from build123d import *

# Parameters (mm, degrees)
BRACKET_PROFILE_DEPTH     = 6
UPRIGHT_ROUNDS_R5_R       = 5
BASE_PLATE_SKETCH_W       = 27
BASE_PLATE_SKETCH_H       = 6
BASE_PLATE_DEPTH          = 12
BASE_PLATE_ROUNDS_R6_R    = 6
BASE_UPRIGHT_FILLETS_R5_R = 5
BASE_SLOT_DEPTH           = 6
PIVOT_HOLES_SKETCH_R      = 2.5
PIVOT_HOLES_2X_5_DEPTH    = 6


with BuildPart() as part:
    # Bracket Profile Sketch → Bracket Profile (new body)
    with BuildSketch(Plane.XY):
        with BuildLine():
            Line((-20, 0), (20, 0))
            Line((20, 0), (20, 18))
            ThreePointArc((20, 18), (15, 23), (10, 18))
            Line((10, 18), (10, 6))
            Line((10, 6), (-10, 6))
            Line((-10, 6), (-10, 18))
            ThreePointArc((-10, 18), (-15, 23), (-20, 18))
            Line((-20, 18), (-20, 0))
        make_face()
    extrude(amount=BRACKET_PROFILE_DEPTH)

    # Upright Rounds R5
    upright_rounds_r5_edges = [part.edges().sort_by_distance(p)[0] for p in [
        (-10, 6, 3),
        (10, 6, 3),
    ]]
    fillet(upright_rounds_r5_edges, radius=UPRIGHT_ROUNDS_R5_R)

    # Base Plate Sketch → Base Plate (add)
    with BuildSketch(Plane.XY.offset(6)):
        with Locations((0, 3)):
            Rectangle(BASE_PLATE_SKETCH_W, BASE_PLATE_SKETCH_H)
    extrude(amount=BASE_PLATE_DEPTH)

    # Base Plate Rounds R6
    base_plate_rounds_r6_edges = [part.edges().sort_by_distance(p)[0] for p in [
        (-13.5, 3, 18),
        (13.5, 3, 18),
    ]]
    fillet(base_plate_rounds_r6_edges, radius=BASE_PLATE_ROUNDS_R6_R)

    # Base-Upright Fillets R5
    base_upright_fillets_r5_edges = [part.edges().sort_by_distance(p)[0] for p in [
        (-13.5, 3, 6),
        (13.5, 3, 6),
    ]]
    fillet(base_upright_fillets_r5_edges, radius=BASE_UPRIGHT_FILLETS_R5_R)

    # Base Slot Sketch → Base Slot (cut)
    with BuildSketch(Plane(origin=(0, 6, 0), x_dir=(1, 0, 0), z_dir=(0, 1, 0))):
        with BuildLine():
            Line((-7.5, -9), (7.5, -9))
            ThreePointArc((7.5, -9), (10.5, -12), (7.5, -15))
            Line((7.5, -15), (-7.5, -15))
            ThreePointArc((-7.5, -15), (-10.5, -12), (-7.5, -9))
        make_face()
    extrude(amount=-BASE_SLOT_DEPTH, mode=Mode.SUBTRACT)

    # Pivot Holes Sketch → Pivot Holes 2xØ5 (cut)
    with BuildSketch(Plane.XY.offset(6)):
        with Locations((-15, 18)):
            Circle(PIVOT_HOLES_SKETCH_R)
        with Locations((15, 18)):
            Circle(PIVOT_HOLES_SKETCH_R)
    extrude(amount=-PIVOT_HOLES_2X_5_DEPTH, mode=Mode.SUBTRACT)


solid = part.part
For this review, take the finished solid that the model builds, in its own axes (mm). A direction names the side the tool comes from. Round coordinates to 2 decimals unless told otherwise and drop trailing zeros. Order: outer loops, then holes, each group sorted by start corner. A loop starts at its lowest first (then second) coordinate and runs counter-clockwise, first axis right, second up. Notation, with made-up numbers: (-33, 89) -> (-12, 89) arc R19 ccw to (-12, 110) -> close; hole circle Ø8 at (76, -39). An arc over 180 degrees is marked (long way). Write item = value, one per line. Start each with the question number.
1) Take a section at B-B on x = 15. State the section outline as (y, z) points, plus the area to 3 significant figures.
2) The part is to be moulded in two halves that separate along Z. For faces 1 (the face through (0, 3, 15)), 2 (the face through (-14.93, 3.04, 7.5)), 3 (the face through (0, 6, 7)), say which applies: +Z half, -Z half, draft (parallel to the pull), parting line (faces both ways), or undercut.
3) Take a section at C-C on y = 15. State the section outline as (x, z) points, plus the area to 3 significant figures.
4) To check wall thickness, follow line 1 (Y direction, x = 15, z = 2.85); line 2 (X direction, y = 20, z = 3); line 3 (Z direction, x = -8, y = 6.5). State the ranges of each line that lie inside material, in increasing order. Write a range as from..to.
5) Take a section at A-A on z = 4.75. State the section outline as (x, y) points.
6) Insertion check: pin 1 (9 mm diameter, centred on x = 1.5, z = 5.5, fed in from +Y); pin 2 (8 mm diameter, centred on x = -16, y = 15, fed in from +Z); pin 3 (0.8 mm diameter, centred on y = 3.5, z = 11.5, fed in from +X). Each pin has a flat end and moves straight along its axis. Give the tip position at first contact, or say it passes through.
7) Take a section at D-D on x = 6. State the section outline as (y, z) points, plus the area to 3 significant figures.
8) Tool access review of faces 4 (the face through (-10.5, 3, 12.1)), 5 (the face through (-13.5, 3, 11.5)), 6 (the face through (-8, 7, 3)): name each direction out of +Z, -Z, +X, -X, +Y, -Y from which nothing blocks a thin tool from reaching the whole face with its end or side.
Verdict:
q1.outline = (0, 0) -> (15.5, 0) -> (15.5, 6) -> (6, 6) -> (6, 7.43) -> (0, 7.43) -> close; (20.5, 0) -> (23, 0) -> (23, 6) -> (20.5, 6) -> close
q1.area = 117 mm2
q2.face_1 = undercut
q2.face_2 = +Z half
q2.face_3 = draft
q3.outline = (-20, 0) -> (-10, 0) -> (-10, 6) -> (-20, 6) -> close; (10, 0) -> (20, 0) -> (20, 6) -> (10, 6) -> close
q3.area = 120 mm2
q4.line_1 = 0..15.5, 20.5..23
q4.line_2 = -19.58..-16.5, -13.5..-10.42, 10.42..13.5, 16.5..19.58
q4.line_3 = 0..6
q5.outline = (-20, 0) -> (20, 0) -> (20, 18) arc R5 ccw to (10, 18) -> (10, 11) arc R5 cw to (5, 6) -> (-5, 6) arc R5 cw to (-10, 11) -> (-10, 18) arc R5 ccw to (-20, 18) -> close; hole circle Ø5 at (-15, 18); hole circle Ø5 at (15, 18)
q6.pin_1 = 6.1
q6.pin_2 = 6
q6.pin_3 = 13.5
q7.outline = (0, 0) -> (6.1, 0) -> (6.1, 6) -> (6, 6) -> (6, 9) -> (0, 9) -> close; (0, 15) -> (6, 15) -> (6, 18) -> (0, 18) -> close
q7.area = 72.6 mm2
q8.face_4 = +Y, -Y
q8.face_5 = +Z, -X, +Y, -Y
q8.face_6 = +Z, -Z, +Y
